Work out the finished part from the listing and answer in its coordinate system (mm). Face numbers are marked on the shaded views. A direction names the side the tool comes from. Round coordinates to 2 decimals unless told otherwise and drop trailing zeros. Loops run counter-clockwise (first coordinate to the right, second up) from the corner with the lowest first, then second, coordinate; pieces in that order, holes last. Notation, with made-up numbers: (-16.5, 47) - (13.5, 47) arc R22 cw to (13.5, 55) - close; hole circle Ø3 at (49, 16.5). An arc over 180 degrees is marked (long way). Return JSON: item names as keys, results as strings.
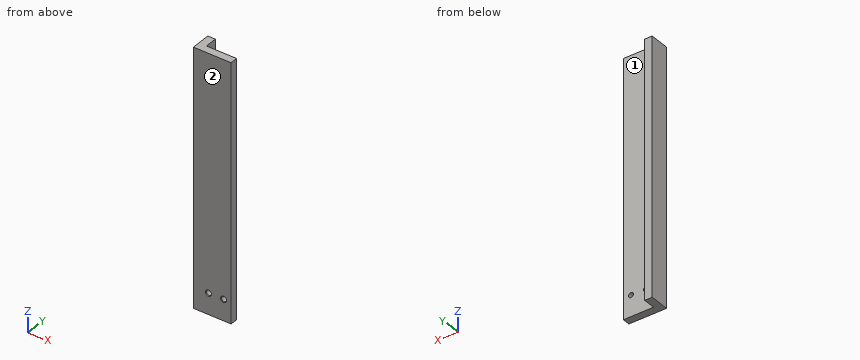
from build123d import *

# Parameters (mm, degrees)
EXTRUDE_1_DEPTH              = 170
HOLE_WIZARD_M4_1_D           = 3.3
HOLE_WIZARD_M4_1_CSINK_D     = 4.05
HOLE_WIZARD_M4_1_CSINK_ANGLE = 90


with BuildPart() as part:
    # 草图1 → 凸台-拉伸1 (new body)
    with BuildSketch(Plane.XY):
        Polygon((0, 0), (0, 13), (5, 13), (5, 5), (25, 5), (25, 0), align=None)
    extrude(amount=EXTRUDE_1_DEPTH)

    # M4 螺纹孔1 (through all)
    with Locations(Plane(origin=(10, 0, 14), x_dir=(-1, 0, 0), z_dir=(0, -1, 0))):
        with Locations((0, 0), (-10, 0)):
            CounterSinkHole(HOLE_WIZARD_M4_1_D / 2, HOLE_WIZARD_M4_1_CSINK_D / 2, counter_sink_angle=HOLE_WIZARD_M4_1_CSINK_ANGLE)


solid = part.part
1) Section C-C (z = 45) is taken. Give the vertices of the cut face in (x, y).
Verdict:
{"outline": "(0, 0) - (25, 0) - (25, 5) - (5, 5) - (5, 13) - (0, 13) - close"}
2) A flat-ended cylindrical pin translates along its axis: pin 1 (1 mm diameter, centred on x = 20.5, z = 113.5, fed in from +Y). Find the tip coordinate at first contact, or state that the pin passes through.
Verdict:
{"pin 1": "stops at y = 5"}
3) A tool of negligible diameter and unlimited length cuts with its end or side. For the marked faces 1 and 2, from which of +Z, -Z, +X, -X, +Y, -Y can it reach the whole face along a straight path? Write none if from no direction.
Verdict:
{"face 1": "+Z, -Z, +X, +Y", "face 2": "+Z, -Z, +X, -X, -Y"}
4) Section D-D (y = 10.25) is taken. Give the vertices of the cut face in (x, z).
Verdict:
{"outline": "(0, 0) - (5, 0) - (5, 170) - (0, 170) - close"}
5) Section B-B (z = 14) is taken. Give the vertices of the cut face in (x, y) (3 decimals), and give its area (3 significant figures).
Verdict:
{"outline": "(0, 0) - (7.975, 0) - (8.35, 0.375) - (8.35, 5) - (5, 5) - (5, 13) - (0, 13) - close; (11.65, 0.375) - (12.025, 0) - (17.975, 0) - (18.35, 0.375) - (18.35, 5) - (11.65, 5) - close; (21.65, 0.375) - (22.025, 0) - (25, 0) - (25, 5) - (21.65, 5) - close", "area": "132 mm2"}
6) Section A-A (x = 20) is taken. Give the vertices of the cut face in (y, z) (3 decimals).
Verdict:
{"outline": "(0, 0) - (5, 0) - (5, 12.35) - (0.375, 12.35) - (0, 11.975) - close; (0, 16.025) - (0.375, 15.65) - (5, 15.65) - (5, 170) - (0, 170) - close"}
7) Find the intervals of material crossed by L1, parallel to X at y = 2.9, z = 14; L2, parallel to Z at x = 20, y = 1.4; L3, parallel to Y at x = 12.5, z = 138.5, in increasing order.
Verdict:
{"L1": "x = 0 to 8.35, 11.65 to 18.35, 21.65 to 25", "L2": "z = 0 to 12.35, 15.65 to 170", "L3": "y = 0 to 5"}
